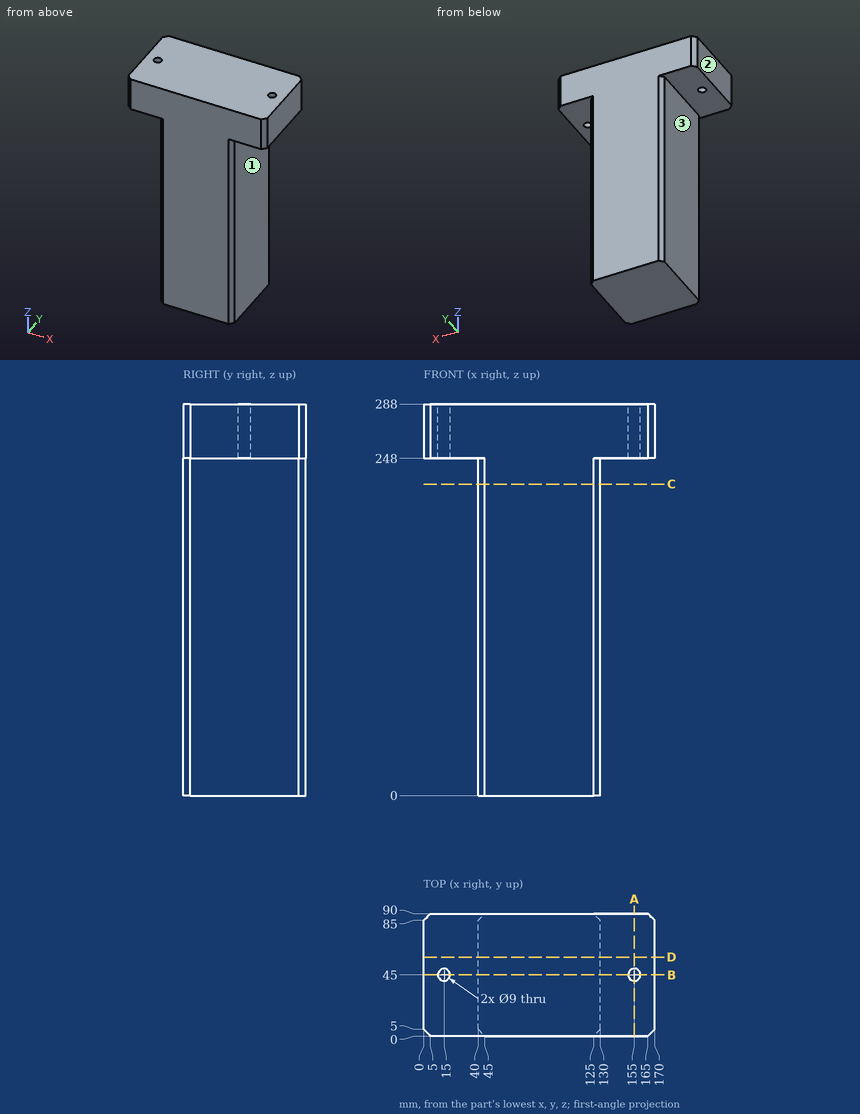
Here's the drawing with two shaded views (mm, measured from the low corner). I have some questions. A direction names the side the tool comes from. Coordinates: 2 decimals unless noted, no trailing zeros. Loops run counter-clockwise (first coordinate to the right, second up) from the corner with the lowest first, then second, coordinate; pieces in that order, holes last. Notation, with made-up numbers: M 64,75 L 112,75 A20 ccw 112,107 Z; hole C -27.5,12.5 d5. An arc over 180 degrees is marked long. Put each result on its own line as item: value. Start each with the question number.
(1) I need wall thicknesses on probe 1 along Y at (x, z) = (15, 259.5); probe 2 along Z at (x, y) = (33, 32); probe 3 along Y at (x, z) = (12.5, 256). Which ranges of each line are inside material? Lowest first, please.
(2) Will these pins go through, and if not, where does the flat tip stop? pin 1 Ø6 at (x, z) = (95, 61) entering from -Y; pin 2 Ø22.5 at (x, y) = (157, 60.5) entering from -Z; pin 3 Ø8 at (x, y) = (15, 45) entering from -Z (3 decimals); pin 4 Ø6 at (y, z) = (75, 64.5) entering from +X.
(3) Imagine slicing it at B-B on y = 45. List the corners of the cut face in (x, z) for me.
(4) Imagine slicing it at A-A on x = 155. List the corners of the cut face in (y, z) for me.
(5) Imagine slicing it at D-D on y = 58. List the corners of the cut face in (x, z) for me, and give its area (3 significant figures).
(6) Which directions (+Z, -Z, +X, -X, +Y, -Y) give clear straight access to the entire face, cutting with the end or side of a thin tool? Please do the marked faces 1, 2 and 3.
(7) Imagine slicing it at C-C on z = 229. List the corners of the cut face in (x, y) for me.
Worked answers:
1. probe 1: y = 0 to 40.5, 49.5 to 90
1. probe 2: z = 248 to 288
1. probe 3: y = 0 to 41.26, 48.74 to 90
2. pin 1: stops at y = 0
2. pin 2: stops at z = 248
2. pin 3: passes through
2. pin 4: stops at x = 130
3. outline: M 0,248 L 10.5,248 L 10.5,288 L 0,288 Z; M 19.5,248 L 40,248 L 40,0 L 130,0 L 130,248 L 150.5,248 L 150.5,288 L 19.5,288 Z; M 159.5,248 L 170,248 L 170,288 L 159.5,288 Z
4. outline: M 0,248 L 40.5,248 L 40.5,288 L 0,288 Z; M 49.5,248 L 90,248 L 90,288 L 49.5,288 Z
5. outline: M 0,248 L 40,248 L 40,0 L 130,0 L 130,248 L 170,248 L 170,288 L 0,288 Z
5. area: 29,100 mm2
6. face 1: -Z, +X, +Y, -Y
6. face 2: +Z, -Z, -X, +Y, -Y
6. face 3: -Z, -X, +Y, -Y
7. outline: M 40,5 L 45,0 L 125,0 L 130,5 L 130,85 L 125,90 L 45,90 L 40,85 Z
